Source: CAD feature listing. Evaluate the final solid. Frame: model axes, mm. Face numbers are marked on the shaded views. A direction names the side the tool comes from. Round coordinates to 2 decimals unless told otherwise and drop trailing zeros. Write each loop counter-clockwise with the first axis right and the second up, starting at its lowest first coordinate (ties: lowest second). Pieces come first, ordered by that corner, then holes. Notation, with made-up numbers: M 68.25,51 L 110.25,51 A14 cw 110.25,78 Z; hole C 14.5,7 d8. An arc over 180 degrees is marked long. Answer in a Markdown table with one row per item.
from build123d import *

# Parameters (mm, degrees)
OVAL_BASE_FLANGE_DEPTH           = 4.4
RAISED_OVAL_BOSS_DEPTH           = 11.6
OVAL_POCKET_R5_DEPTH             = 5
COUNTERBORE_SKETCH_R             = 3.5
MOUNTING_HOLE_COUNTERBORES_DEPTH = 1
MOUNTING_HOLES_SKETCH_R          = 1.7
MOUNTING_HOLES_3_4_DEPTH         = 7
THROUGH_SLOT_SKETCH_R            = 2.5
POCKET_THROUGH_SLOT_DEPTH        = 15
BOSS_ROOT_FILLET_R1_R            = 1


with BuildPart() as part:
    # Base Flange Sketch → Oval Base Flange (new body)
    with BuildSketch(Plane(origin=(0, 0, 0), x_dir=(1, 0, 0), z_dir=(0, 1, 0))):
        with BuildLine():
            Line((11.25, -18), (-11.25, -18))
            ThreePointArc((-11.25, -18), (-29.25, 0), (-11.25, 18))
            Line((-11.25, 18), (11.25, 18))
            ThreePointArc((11.25, 18), (29.25, 0), (11.25, -18))
        make_face()
    extrude(amount=OVAL_BASE_FLANGE_DEPTH)

    # Oval Boss Sketch → Raised Oval Boss (add)
    with BuildSketch(Plane(origin=(0, 4.4, 0), x_dir=(1, 0, 0), z_dir=(0, 1, 0))):
        with BuildLine():
            Line((-11.25, 7.6), (11.25, 7.6))
            ThreePointArc((11.25, 7.6), (18.85, 0), (11.25, -7.6))
            Line((11.25, -7.6), (-11.25, -7.6))
            ThreePointArc((-11.25, -7.6), (-18.85, 0), (-11.25, 7.6))
        make_face()
    extrude(amount=RAISED_OVAL_BOSS_DEPTH)

    # Oval Pocket Sketch → Oval Pocket R5 (cut)
    with BuildSketch(Plane(origin=(0, 16, 0), x_dir=(1, 0, 0), z_dir=(0, 1, 0))):
        with BuildLine():
            Line((-11.25, 5), (11.25, 5))
            ThreePointArc((11.25, 5), (16.25, 0), (11.25, -5))
            Line((11.25, -5), (-11.25, -5))
            ThreePointArc((-11.25, -5), (-16.25, 0), (-11.25, 5))
        make_face()
    extrude(amount=-OVAL_POCKET_R5_DEPTH, mode=Mode.SUBTRACT)

    # Counterbore Sketch → Mounting Hole Counterbores (cut)
    with BuildSketch(Plane(origin=(0, 4.4, 0), x_dir=(1, 0, 0), z_dir=(0, 1, 0))):
        with Locations(Location((-11.25, 13, 0), (0, 0, 270))):
            Circle(COUNTERBORE_SKETCH_R)
        with Locations(Location((11.25, 13, 0), (0, 0, 90))):
            Circle(COUNTERBORE_SKETCH_R)
        with Locations(Location((11.25, -13, 0), (0, 0, 270))):
            Circle(COUNTERBORE_SKETCH_R)
        with Locations(Location((-11.25, -13, 0), (0, 0, 90))):
            Circle(COUNTERBORE_SKETCH_R)
        with Locations(Location((-24.25, 0, 0), (0, 0, 270))):
            Circle(COUNTERBORE_SKETCH_R)
        with Locations(Location((24.25, 0, 0), (0, 0, 90))):
            Circle(COUNTERBORE_SKETCH_R)
    extrude(amount=-MOUNTING_HOLE_COUNTERBORES_DEPTH, mode=Mode.SUBTRACT)

    # Mounting Holes Sketch → Mounting Holes Ø3.4 (cut)
    with BuildSketch(Plane(origin=(0, 3.4, 0), x_dir=(1, 0, 0), z_dir=(0, 1, 0))):
        with Locations(Location((-11.25, 13, 0), (0, 0, 270))):
            Circle(MOUNTING_HOLES_SKETCH_R)
        with Locations(Location((11.25, 13, 0), (0, 0, 270))):
            Circle(MOUNTING_HOLES_SKETCH_R)
        with Locations(Location((11.25, -13, 0), (0, 0, 270))):
            Circle(MOUNTING_HOLES_SKETCH_R)
        with Locations(Location((-11.25, -13, 0), (0, 0, 270))):
            Circle(MOUNTING_HOLES_SKETCH_R)
        with Locations(Location((-24.25, 0, 0), (0, 0, 270))):
            Circle(MOUNTING_HOLES_SKETCH_R)
        with Locations(Location((24.25, 0, 0), (0, 0, 270))):
            Circle(MOUNTING_HOLES_SKETCH_R)
    extrude(amount=-MOUNTING_HOLES_3_4_DEPTH, mode=Mode.SUBTRACT)

    # Through Slot Sketch → Pocket Through Slot (cut)
    with BuildSketch(Plane(origin=(0, 11, 0), x_dir=(1, 0, 0), z_dir=(0, 1, 0))):
        with Locations(Location((-11.25, 0, 0), (0, 0, 270))):
            Circle(THROUGH_SLOT_SKETCH_R)
        with Locations(Location((11.25, 0, 0), (0, 0, 270))):
            Circle(THROUGH_SLOT_SKETCH_R)
    extrude(amount=-POCKET_THROUGH_SLOT_DEPTH, mode=Mode.SUBTRACT)

    # Boss Root Fillet R1
    boss_root_fillet_r1_edges = [part.edges().sort_by_distance(p)[0] for p in [
        (-29.25, 4.4, 0),
        (-18.85, 4.4, 0),
        (0, 4.4, 18),
        (0, 4.4, 7.6),
        (18.85, 4.4, 0),
        (0, 4.4, -7.6),
        (29.25, 4.4, 0),
        (0, 4.4, -18),
    ]]
    fillet(boss_root_fillet_r1_edges, radius=BOSS_ROOT_FILLET_R1_R)


solid = part.part
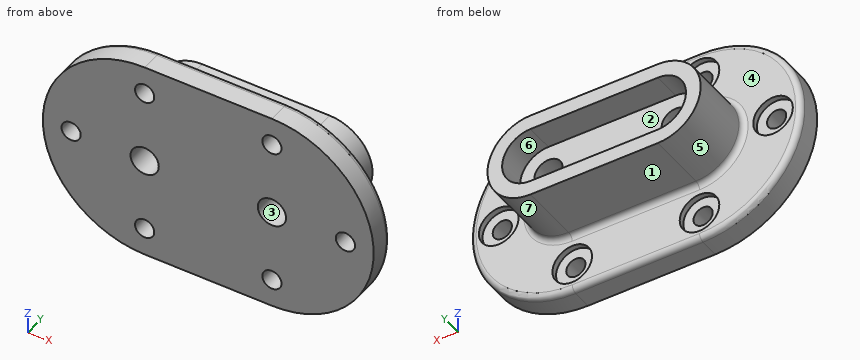
Q1. Section A-A (y = 7.75). Return loops of the section in (x, z).
Solutions:
| item | result |
|---|---|
| outline | M -11.25,-7.6 L 11.25,-7.6 A7.6 ccw 11.25,7.6 L -11.25,7.6 A7.6 ccw Z; hole C -11.25,0 d5; hole C 11.25,0 d5 |
Q2. Section C-C (y = 2.75). State how many separate pieces and enclosed holes the cut face has, and give its area (3 significant figures).
Solutions:
| item | result |
|---|---|
| separate pieces | 1 |
| enclosed holes | 8 |
| area | 1,730 mm2 |
Q3. Section B-B (x = 7). Return loops of the section in (y, z).
Solutions:
| item | result |
|---|---|
| outline | M 0,-18 L 3.4,-18 A1 ccw 4.4,-17 L 4.4,-8.6 A1 cw 5.4,-7.6 L 16,-7.6 L 16,-5 L 11,-5 L 11,5 L 16,5 L 16,7.6 L 5.4,7.6 A1 cw 4.4,8.6 L 4.4,17 A1 ccw 3.4,18 L 0,18 Z |
Q4. Pull-direction query (X, two-part tool) for the marked faces 4, 5, 6 and 7; classes: pulls with the +X half, pulls with the -X half, needs draft (parallel to the pull), parting line crosses it, or undercut.
Solutions:
| item | result |
|---|---|
| face 4 | needs draft |
| face 5 | pulls with the -X half |
| face 6 | undercut |
| face 7 | pulls with the +X half |
Q5. Material intervals for probe 1 along X at (y, z) = (2.5, 0); probe 2 along Z at (x, y) = (2, 14); probe 3 along X at (y, z) = (1.3, 13), sorted ascending.
Solutions:
| item | result |
|---|---|
| probe 1 | x = -29.25 to -25.95, -22.55 to -13.75, -8.75 to 8.75, 13.75 to 22.55, 25.95 to 29.25 |
| probe 2 | z = -7.6 to -5, 5 to 7.6 |
| probe 3 | x = -23.7 to -12.95, -9.55 to 9.55, 12.95 to 23.7 |
Q6. Contact query for flat-ended pins moving along their axis: pin 1 Ø2 at (x, y) = (4, 5) entering from +Z; pin 2 Ø5.5 at (x, z) = (-24.25, 0) entering from +Y; pin 3 Ø2 at (y, z) = (10.5, 3) entering from -X; pin 4 Ø2 at (x, z) = (-11.25, -13) entering from -Y. Output: stop coordinate, or through.
Solutions:
| item | result |
|---|---|
| pin 1 | stops at z = 17.8 |
| pin 2 | stops at y = 3.4 |
| pin 3 | stops at x = -18.58 |
| pin 4 | passes through |
Q7. Access query for the marked faces 1, 2 and 3. Directions: +Z, -Z, +X, -X, +Y, -Y. A direction counts if a zero-diameter tool reaches every point of the face in a straight line with its end or side. Return the directions, or none.
Solutions:
| item | result |
|---|---|
| face 1 | -Z, +X, -X, +Y |
| face 2 | +Y |
| face 3 | +Y, -Y |
